Part model, mm, in its own coordinate system. A direction names the side the tool comes from. Round coordinates to 2 decimals unless told otherwise and drop trailing zeros. Write each loop counter-clockwise with the first axis right and the second up, starting at its lowest first coordinate (ties: lowest second). Pieces come first, ordered by that corner, then holes. Notation, with made-up numbers: (-24, 52) -> (10, 52) arc R23 cw to (10, 63) -> close; hole circle Ø8 at (81, 15.25). An arc over 180 degrees is marked (long way). Return JSON: item names as keys, results as strings. Group by question number.
(1) Saw through at D-D (z = 77). List the corners of the cut face in (x, y).
(2) Saw through at C-C (y = 0). List the corners of the cut face in (x, z).
(3) Saw through at B-B (x = 0). State how many separate pieces and enclosed holes the cut face has, plus the area to 3 significant figures.
(4) Drill centre lines: L1, parallel to X at y = 1, z = 20; L2, parallel to Z at x = 0.75, y = 4; L3, parallel to Z at x = 1.25, y = 3.5. Where is each one in solid material? Low to high. Write a range as from..to.
(5) Drop a flat-ended pin along its axis: pin 1 Ø5.5 at (x, z) = (0, 20) entering from -Y. Give the stop position or say it passes through.
(6) Saw through at A-A (z = 5). List the corners of the cut face in (x, y).
(7) Tool access for faces 1 (the cylindrical face through (-0.596, 2.685, 70.748)), 2 (the flat face through (-3, 5, 18)), 3 (the cylindrical face through (-3, 0, 96)): list every direction of +Z, -Z, +X, -X, +Y, -Y with a clear straight run to the whole face (end or side of a thin tool).
(8) Mould opens along Z. For faces 4 (the cylindrical face through (0, 0, 17)), 5 (the flat face through (0, 0, 104)), 6 (the flat face through (-3, -5, 18)), 7 (the cylindrical face through (0, 0, 2)) say: +Z half, -Z half, draft (parallel to the pull), parting line (faces both ways), or undercut.
from build123d import *

# Parameters (mm, degrees)
SKETCH1_W           = 10
SKETCH1_H           = 10
BOSS_EXTRUDE1_DEPTH = 36
SKETCH2_R           = 4
BOSS_EXTRUDE2_DEPTH = 2
SKETCH3_R           = 3
BOSS_EXTRUDE3_DEPTH = 66
SKETCH4_R           = 3
CUT_EXTRUDE1_DEPTH  = 50
CHAMFER1_SIZE       = 0.5
CHAMFER2_SIZE       = 0.5
SKETCH6_W           = 5
SKETCH6_H           = 36


with BuildPart() as part:
    # Sketch1 → Boss-Extrude1 (new body)
    with BuildSketch(Plane.XY):
        Rectangle(SKETCH1_W, SKETCH1_H)
    extrude(amount=BOSS_EXTRUDE1_DEPTH)

    # Sketch2 → Boss-Extrude2 (add)
    with BuildSketch(Plane.XY.offset(36)):
        Circle(SKETCH2_R)
    extrude(amount=BOSS_EXTRUDE2_DEPTH)

    # Sketch3 → Boss-Extrude3 (add)
    with BuildSketch(Plane.XY.offset(38)):
        Circle(SKETCH3_R)
    extrude(amount=BOSS_EXTRUDE3_DEPTH)

    # Sketch4 → Cut-Extrude1 (cut)
    with BuildSketch(Plane(origin=(0, 5, 0), x_dir=(1, 0, 0), z_dir=(0, 1, 0))):
        with Locations(Location((0, -5, 0), (0, 0, 270))):
            Circle(SKETCH4_R)
        with Locations(Location((0, -20, 0), (0, 0, 270))):
            Circle(SKETCH4_R)
    extrude(amount=-CUT_EXTRUDE1_DEPTH, mode=Mode.SUBTRACT)

    # Chamfer1
    chamfer1_edges = [part.edges().sort_by_distance(p)[0] for p in [
        (5, -5, 18),
        (-5, -5, 18),
        (-5, 5, 18),
        (5, 5, 18),
    ]]
    chamfer(chamfer1_edges, length=CHAMFER1_SIZE)

    # Chamfer2
    chamfer2_edges = [part.edges().sort_by_distance(p)[0] for p in [
        (-3, 0, 104),
    ]]
    chamfer(chamfer2_edges, length=CHAMFER2_SIZE)

    # Sketch6 → Cut-Revolve1 (revolve, cut)
    with BuildSketch(Plane(origin=(0, 0, 0), x_dir=(1, 0, 0), z_dir=(0, 1, 0))):
        with Locations((5.25, -71)):
            Rectangle(SKETCH6_W, SKETCH6_H)
    revolve(axis=Axis((0, 0, 103.5), (0, 0, -1)), mode=Mode.SUBTRACT)


solid = part.part
Computed values:
{
 "1": {"outline": "circle Ø5.5 at (0, 0)"},
 "2": {"outline": "(-5, 0) -> (5, 0) -> (5, 36) -> (4, 36) -> (4, 38) -> (3, 38) -> (3, 53) -> (2.75, 53) -> (2.75, 89) -> (3, 89) -> (3, 103.5) -> (2.5, 104) -> (-2.5, 104) -> (-3, 103.5) -> (-3, 89) -> (-2.75, 89) -> (-2.75, 53) -> (-3, 53) -> (-3, 38) -> (-4, 38) -> (-4, 36) -> (-5, 36) -> close; hole circle Ø6 at (0, 5); hole circle Ø6 at (0, 20)"},
 "3": {"separate pieces": "3", "enclosed holes": "0", "area": "634 mm2"},
 "4": {"L1": "-5..-3, 3..5", "L2": "0..2.1, 7.9..17.1, 22.9..36", "L3": "0..2.27, 7.73..17.27, 22.73..38"},
 "5": {"pin 1": "through"},
 "6": {"outline": "(-5, -4.5) -> (-4.5, -5) -> (-3, -5) -> (-3, 5) -> (-4.5, 5) -> (-5, 4.5) -> close; (3, -5) -> (4.5, -5) -> (5, -4.5) -> (5, 4.5) -> (4.5, 5) -> (3, 5) -> close"},
 "7": {"face 1": "none", "face 2": "+Z, -Z, +X, -X, +Y", "face 3": "+Z"},
 "8": {"face 4": "undercut", "face 5": "+Z half", "face 6": "draft", "face 7": "undercut"}
}
